from build123d import *

# Parameters (mm, degrees)
SKETCH1_R                                           = 5
BOSS_EXTRUDE1_DEPTH                                 = 10
SKETCH2_R                                           = 13
BOSS_EXTRUDE2_DEPTH                                 = 5
SKETCH3_R                                           = 4
BOSS_EXTRUDE3_DEPTH                                 = 20
SKETCH4_R                                           = 2.5
CUT_EXTRUDE1_DEPTH                                  = 30
CBORE_FOR_M3_HEX_SOCKET_HEAD_CAP_SCREW1_D           = 3.4
CBORE_FOR_M3_HEX_SOCKET_HEAD_CAP_SCREW1_CBORE_D     = 6.5
CBORE_FOR_M3_HEX_SOCKET_HEAD_CAP_SCREW1_CBORE_DEPTH = 3.4
CIRPATTERN1_COUNT                                   = 3
CUT_EXTRUDE2_DEPTH                                  = 42.024382994
CHAMFER1_SIZE                                       = 0.5


with BuildPart() as part:
    # Sketch1 → Boss-Extrude1 (new body)
    with BuildSketch(Plane.XY):
        Circle(SKETCH1_R)
    extrude(amount=BOSS_EXTRUDE1_DEPTH)

    # Sketch2 → Boss-Extrude2 (add)
    with BuildSketch(Plane.XY.offset(10)):
        Circle(SKETCH2_R)
    extrude(amount=BOSS_EXTRUDE2_DEPTH)

    # Sketch3 → Boss-Extrude3 (add)
    with BuildSketch(Plane.XY.offset(15)):
        Circle(SKETCH3_R)
    extrude(amount=BOSS_EXTRUDE3_DEPTH)

    # Sketch4 → Cut-Extrude1 (cut)
    with BuildSketch(Plane.XY.offset(35)):
        Circle(SKETCH4_R)
    extrude(amount=-CUT_EXTRUDE1_DEPTH, mode=Mode.SUBTRACT)

    # CBORE for M3 Hex Socket Head Cap Screw1 (through all)
    with Locations(Plane.XY.offset(15)):
        with Locations((9, 0)):
            cbore_for_m3_hex_socket_head_cap_screw1 = CounterBoreHole(CBORE_FOR_M3_HEX_SOCKET_HEAD_CAP_SCREW1_D / 2, CBORE_FOR_M3_HEX_SOCKET_HEAD_CAP_SCREW1_CBORE_D / 2, CBORE_FOR_M3_HEX_SOCKET_HEAD_CAP_SCREW1_CBORE_DEPTH)

    # CirPattern1: CBORE for M3 Hex Socket Head Cap Screw1 ×3 about axis
    cirpattern1_axis = Axis((0, 0, 0), (0, 0, 1))
    for i in range(1, CIRPATTERN1_COUNT):
        add(cbore_for_m3_hex_socket_head_cap_screw1.rotate(cirpattern1_axis, i * 360 / CIRPATTERN1_COUNT), mode=Mode.SUBTRACT)

    # Sketch7 → Cut-Extrude2 (cut, through all)
    with BuildSketch(Plane(origin=(4, 0, 0), x_dir=(0, 0, -1), z_dir=(1, 0, 0))):
        with BuildLine():
            Line((-27, 1), (-19, 1))
            ThreePointArc((-19, 1), (-18, 0), (-19, -1))
            Line((-19, -1), (-27, -1))
            ThreePointArc((-27, -1), (-28, 0), (-27, 1))
        make_face()
    extrude(amount=-CUT_EXTRUDE2_DEPTH, mode=Mode.SUBTRACT)

    # Chamfer1
    chamfer1_edges = [part.edges().sort_by_distance(p)[0] for p in [
        (-4, 0, 35),
        (-2.5, 0, 35),
        (-5, 0, 0),
        (-13, 0, 10),
        (-13, 0, 15),
    ]]
    chamfer(chamfer1_edges, length=CHAMFER1_SIZE)


solid = part.part
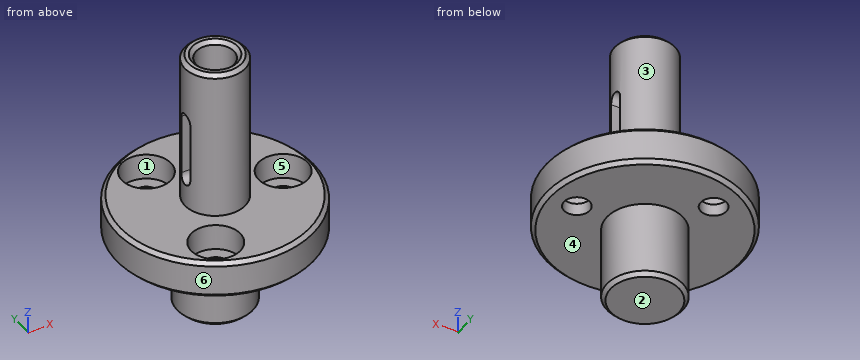
Geometry check sheet. Reference: the model listing, model coordinates, mm. Face numbers are marked on the shaded views. A direction names the side the tool comes from. Round coordinates to 2 decimals unless told otherwise and drop trailing zeros. Write each loop counter-clockwise with the first axis right and the second up, starting at its lowest first coordinate (ties: lowest second). Pieces come first, ordered by that corner, then holes. Notation, with made-up numbers: (33.25, -16.5) -> (37.25, -16.5) arc R19 ccw to (37.25, 8.5) -> close; hole circle Ø7 at (1.25, 88). An arc over 180 degrees is marked (long way). One line per item, written item: value. Start each with the question number.
(1) Cross-section at A-A, the plane x = 0. Record the cut outline in (y, z), and give its area (3 significant figures).
(2) Draft check along Y on the marked faces 1, 2 and 3. Enter one of: +Y half, -Y half, draft (parallel to the pull), parting line (faces both ways), or undercut.
(3) Access from +Z, -Z, +X, -X, +Y, -Y to the whole of each face (thin tool, end or side, straight path). Record for the marked faces 4, 5 and 6.
(4) Go/stop test with flat-tipped pins: pin 1 Ø5.5 at (x, y) = (9, 0) entering from +Z; pin 2 Ø7 at (x, y) = (-3, -7) entering from +Z; pin 3 Ø7.5 at (x, y) = (-1.5, 4) entering from +Z; pin 4 Ø1 at (x, z) = (0.5, 16.5) entering from +Y. Record where each tip stops, or that it passes through.
(5) Cross-section at D-D, the plane z = 7. Record the cut outline in (x, y), and give its area (3 significant figures).
(6) Scan lines: line 1 (Y direction, x = -4.5, z = 12.7); line 2 (Y direction, x = 0, z = 12.5); line 3 (Y direction, x = -4.5, z = 10.55). Record each from-to range of solid material in increasing order. Write a range as [from, to].
(7) Cross-section at C-C, the plane y = 0. Give the number of separate pieces and of enclosed holes in the cut face, and give its area (3 significant figures).
(8) Cross-section at B-B, the plane z = 13.5. Record the cut outline in (x, y) (3 decimals).
Answer:
1. outline: (-13, 10.5) -> (-12.5, 10) -> (-5, 10) -> (-5, 0.5) -> (-4.5, 0) -> (4.5, 0) -> (5, 0.5) -> (5, 10) -> (12.5, 10) -> (13, 10.5) -> (13, 14.5) -> (12.5, 15) -> (4, 15) -> (4, 34.5) -> (3.5, 35) -> (3, 35) -> (2.5, 34.5) -> (2.5, 5) -> (-2.5, 5) -> (-2.5, 34.5) -> (-3, 35) -> (-3.5, 35) -> (-4, 34.5) -> (-4, 15) -> (-12.5, 15) -> (-13, 14.5) -> close
1. area: 239 mm²
2. face 1: undercut
2. face 2: draft
2. face 3: parting line
3. face 4: -Z
3. face 5: +Z
3. face 6: +Z, -Z
4. pin 1: z = 11.6
4. pin 2: z = 15
4. pin 3: z = 35
4. pin 4: y = 4
5. outline: circle Ø10 at (0, 0); hole circle Ø5 at (0, 0)
5. area: 58.9 mm²
6. line 1: [-12.2, -11.04], [-4.54, 4.54], [11.04, 12.2]
6. line 2: [-13, -2.5], [2.5, 13]
6. line 3: [-12.2, -9.49], [-6.09, 6.09], [9.49, 12.2]
7. separate pieces: 4
7. enclosed holes: 0
7. area: 181 mm²
8. outline: circle Ø26 at (0, 0); hole circle Ø6.5 at (-4.5, -7.794); hole circle Ø6.5 at (-4.5, 7.794); hole circle Ø5 at (0, 0); hole circle Ø6.5 at (9, 0)
